Design review of the part built by this model. Coordinates are the model's own, in mm. Coordinates: 2 decimals unless noted, no trailing zeros. Loops run counter-clockwise (first coordinate to the right, second up) from the corner with the lowest first, then second, coordinate; pieces in that order, holes last. Notation, with made-up numbers: (-18.75, 2.5) -> (8.25, 2.5) arc R34 cw to (8.25, 41.5) -> close; hole circle Ø1 at (4.25, 59). An arc over 180 degrees is marked (long way). Use CSV: the item, a comma, the result in double quotes.
```python
from build123d import *

# Parameters (mm, degrees)
SKETCH1_R           = 7.5
SKETCH1_R_2         = 8.652423936
BOSS_EXTRUDE1_DEPTH = 10


with BuildPart() as part:
    # Sketch1 → Boss-Extrude1 (new body)
    with BuildSketch(Plane.XY):
        Polygon((0, 0), (600, 0), (600, 50), (480, 50), (480, 70), (360, 70), (360, 90), (240, 90), (240, 110), (120, 110), (120, 130), (0, 130), align=None)
        with Locations((60, 110)):
            Circle(SKETCH1_R, mode=Mode.SUBTRACT)
        with Locations((180, 90)):
            Circle(SKETCH1_R_2, mode=Mode.SUBTRACT)
        with Locations((300, 70)):
            Circle(SKETCH1_R, mode=Mode.SUBTRACT)
        with Locations((420, 50)):
            Circle(SKETCH1_R, mode=Mode.SUBTRACT)
        with Locations((540, 30)):
            Circle(SKETCH1_R, mode=Mode.SUBTRACT)
    extrude(amount=BOSS_EXTRUDE1_DEPTH)


solid = part.part
```
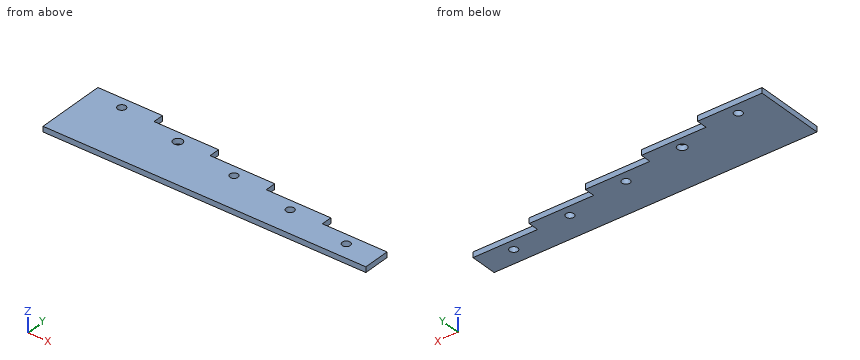
Item 1: Clearance check with flat-ended pins moving along their axes: pin 1 (14 mm diameter, centred on x = 180, y = 90, fed in from +Z); pin 2 (3 mm diameter, centred on y = 58, z = 5.5, fed in from +X); pin 3 (5 mm diameter, centred on x = 271.5, z = 4.5, fed in from +Y). State where each tip first meets the part, or that it passes through.
Checked values:
pin 1,"through"
pin 2,"x = 480"
pin 3,"y = 90"
Item 2: Add section B-B (z = 7.5). Give the boundary of the cut face in (x, y).
Checked values:
outline,"(0, 0) -> (600, 0) -> (600, 50) -> (480, 50) -> (480, 70) -> (360, 70) -> (360, 90) -> (240, 90) -> (240, 110) -> (120, 110) -> (120, 130) -> (0, 130) -> close; hole circle Ø15 at (60, 110); hole circle Ø17.3 at (180, 90); hole circle Ø15 at (300, 70); hole circle Ø15 at (420, 50); hole circle Ø15 at (540, 30)"
Item 3: Add section D-D (x = 263). Give the boundary of the cut face in (y, z), then the cut area to 3 significant figures.
Checked values:
outline,"(0, 0) -> (90, 0) -> (90, 10) -> (0, 10) -> close"
area,"900 mm^2"
Item 4: To check wall thickness, follow line 1 along X through (y, z) = (49, 9.25); line 2 along Y through (x, z) = (420, 5); line 3 along X through (y, z) = (89.5, 6.5). State the ranges of each line that lie inside material, in increasing order.
Checked values:
line 1,"0 to 412.57, 427.43 to 600"
line 2,"0 to 42.5, 57.5 to 70"
line 3,"0 to 171.36, 188.64 to 360"
Item 5: Add section A-A (x = 540). Give the boundary of the cut face in (y, z), then the cut area to 3 significant figures.
Checked values:
outline,"(0, 0) -> (22.5, 0) -> (22.5, 10) -> (0, 10) -> close; (37.5, 0) -> (50, 0) -> (50, 10) -> (37.5, 10) -> close"
area,"350 mm^2"
Item 6: Add section C-C (y = 30). Give the boundary of the cut face in (x, z), then the cut area to 3 significant figures.
Checked values:
outline,"(0, 0) -> (532.5, 0) -> (532.5, 10) -> (0, 10) -> close; (547.5, 0) -> (600, 0) -> (600, 10) -> (547.5, 10) -> close"
area,"5,850 mm^2"
